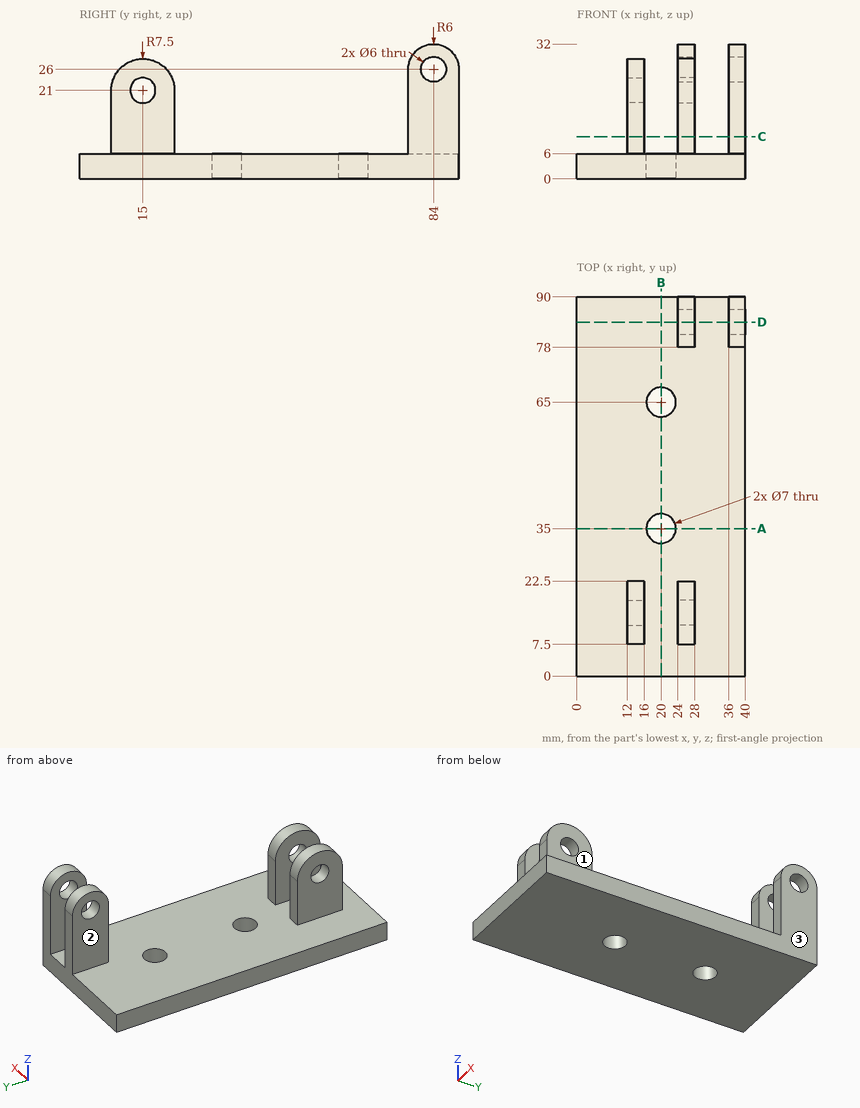
Design review of the part shown in the three views and the two pictorial views. Dimensions are in mm from the part's minimum x, y and z. A direction names the side the tool comes from. Round coordinates to 2 decimals unless told otherwise and drop trailing zeros. Loops run counter-clockwise (first coordinate to the right, second up) from the corner with the lowest first, then second, coordinate; pieces in that order, holes last.
(1) Clearance check with flat-ended pins moving along their axes: P1, Ø4, axis at x = 28.5, y = 22, coming from the +Z side; P2, Ø6, axis at x = 28, y = 69, coming from the +Z side; P3, Ø4.5, axis at y = 13, z = 20, coming from the -X side. State where each tip first meets the part, or that it passes through.
Returned:
P1: stops at z = 26.53
P2: stops at z = 6
P3: stops at x = 12
(2) We need section B-B (x = 20). Give the boundary of the cut face in (y, z), plus the area to 3 significant figures.
Returned:
outline: (0, 0) - (31.5, 0) - (31.5, 6) - (0, 6) - close; (38.5, 0) - (61.5, 0) - (61.5, 6) - (38.5, 6) - close; (68.5, 0) - (90, 0) - (90, 6) - (68.5, 6) - close
area: 456 mm2
(3) Wall thickness on line 1 along Y through (x, z) = (20, 4); line 2 along Y through (x, z) = (26.5, 9); line 3 along Y through (x, z) = (26.5, 21): over which ranges is each line inside the solid? List them lowest first.
Returned:
line 1: y = 0 to 31.5, 38.5 to 61.5, 68.5 to 90
line 2: y = 7.5 to 22.5, 78 to 90
line 3: y = 7.5 to 12, 18 to 22.5, 78 to 90
(4) We need section A-A (y = 35). Give the boundary of the cut face in (x, z), plus the area to 3 significant figures.
Returned:
outline: (0, 0) - (16.5, 0) - (16.5, 6) - (0, 6) - close; (23.5, 0) - (40, 0) - (40, 6) - (23.5, 6) - close
area: 198 mm2
(5) Tool access review of the marked faces 1, 2 and 3: name each direction out of +Z, -Z, +X, -X, +Y, -Y from which nothing blocks a thin tool from reaching the whole face with its end or side.
Returned:
face 1: +Z, +X, +Y, -Y
face 2: +Z, -X, +Y, -Y
face 3: +Z, -Z, +X, +Y, -Y
(6) We need section C-C (z = 10). Give the boundary of the cut face in (x, y).
Returned:
outline: (12, 7.5) - (16, 7.5) - (16, 22.5) - (12, 22.5) - close; (24, 7.5) - (28, 7.5) - (28, 22.5) - (24, 22.5) - close; (24, 78) - (28, 78) - (28, 90) - (24, 90) - close; (36, 78) - (40, 78) - (40, 90) - (36, 90) - close
(7) We need section D-D (y = 84). Give the boundary of the cut face in (x, z), plus the area to 3 significant figures.
Returned:
outline: (0, 0) - (40, 0) - (40, 23) - (36, 23) - (36, 6) - (28, 6) - (28, 23) - (24, 23) - (24, 6) - (0, 6) - close; (24, 29) - (28, 29) - (28, 32) - (24, 32) - close; (36, 29) - (40, 29) - (40, 32) - (36, 32) - close
area: 400 mm2
